The model under review builds one solid part; all positions refer to its coordinate system, in mm. Face numbers are marked on the shaded views. A direction names the side the tool comes from. Coordinates: 2 decimals unless noted, no trailing zeros. Order: outer loops, then holes, each group sorted by start corner. A loop starts at its lowest first (then second) coordinate and runs counter-clockwise, first axis right, second up. Notation, with made-up numbers: M 27.25,4.25 L 38.25,4.25 A33 cw 38.25,43.25 Z; hole C -37.75,70 d1. An arc over 180 degrees is marked long. Answer in a Markdown table with one row per item.
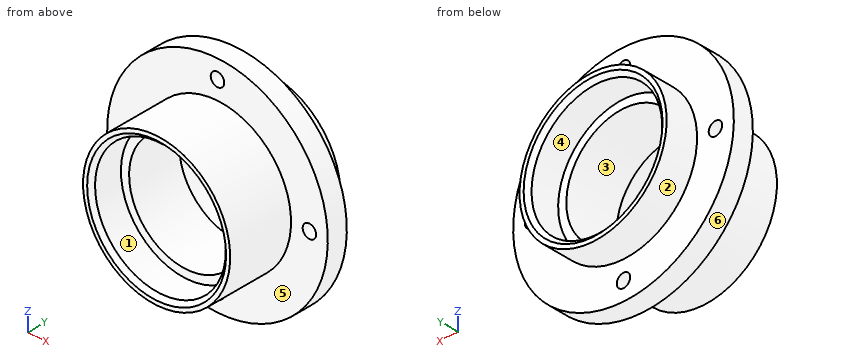
from build123d import *

# Parameters (mm, degrees)
SKETCH1_R             = 18
BOSS_EXTRUDE1_DEPTH   = 8
CUT_EXTRUDE1_REACH    = 28.683
SKETCH2_R             = 16
SKETCH3_R             = 27
BOSS_EXTRUDE2_DEPTH   = 5
BOSS_EXTRUDE3_START   = 16
SKETCH4_R             = 18
BOSS_EXTRUDE3_DEPTH   = 16
SKETCH5_R             = 16
CUT_EXTRUDE2_DEPTH    = 7.8
SKETCH6_R             = 14
CUT_EXTRUDE3_DEPTH    = 44.577517139
M4_TAPPED_HOLE1_D     = 3.3
M4_TAPPED_HOLE1_DEPTH = 11.5
M4_TAPPED_HOLE1_TIP   = 0.991420021
CHAMFER1_SIZE         = 1


with BuildPart() as part:
    # Sketch1 → Boss-Extrude1 (new body)
    with BuildSketch(Plane(origin=(0, 0, 0), x_dir=(1, 0, 0), z_dir=(0, 1, 0))):
        with Locations(Location((0, 0, 0), (0, 0, 270))):
            Circle(SKETCH1_R)
    extrude(amount=BOSS_EXTRUDE1_DEPTH)

    # Sketch2 → Cut-Extrude1 (cut, up to next)
    with BuildSketch(Plane.XZ, mode=Mode.PRIVATE) as cut_extrude1_sk1:
        with Locations(Location((0, 0, 0), (0, 0, 270))):
            Circle(SKETCH2_R)
    cut_extrude1_tool1 = extrude(cut_extrude1_sk1.sketch, amount=-CUT_EXTRUDE1_REACH, mode=Mode.PRIVATE) & part.part
    add(cut_extrude1_tool1.solids().sort_by_distance((0, 0, 0))[0], mode=Mode.SUBTRACT)

    # Sketch3 → Boss-Extrude2 (add)
    with BuildSketch(Plane.XZ):
        with Locations(Location((0, 0, 0), (0, 0, 270))):
            Circle(SKETCH3_R)
    extrude(amount=BOSS_EXTRUDE2_DEPTH)

    # Sketch4 → Boss-Extrude3 (add)
    with BuildSketch(Plane.XZ.offset(5).offset(BOSS_EXTRUDE3_START)):
        with Locations(Location((0, 0, 0), (0, 0, 270))):
            Circle(SKETCH4_R)
    extrude(amount=-BOSS_EXTRUDE3_DEPTH)

    # Sketch5 → Cut-Extrude2 (cut)
    with BuildSketch(Plane.XZ.offset(21)):
        with Locations(Location((0, 0, 0), (0, 0, 270))):
            Circle(SKETCH5_R)
    extrude(amount=-CUT_EXTRUDE2_DEPTH, mode=Mode.SUBTRACT)

    # Sketch6 → Cut-Extrude3 (cut, through all)
    with BuildSketch(Plane(origin=(0, 0, 0), x_dir=(1, 0, 0), z_dir=(0, 1, 0))):
        with Locations(Location((0, 0, 0), (0, 0, 270))):
            Circle(SKETCH6_R)
    extrude(amount=-CUT_EXTRUDE3_DEPTH, mode=Mode.SUBTRACT)

    # M4 Tapped Hole1
    with Locations(Plane(origin=(0, 0, 0), x_dir=(1, 0, 0), z_dir=(0, 1, 0))):
        with Locations((-22.5, 0), (0, 0), (0, 22.5), (22.5, 0), (0, -22.5)):
            Hole(M4_TAPPED_HOLE1_D / 2, depth=M4_TAPPED_HOLE1_DEPTH)
            with Locations((0, 0, -(M4_TAPPED_HOLE1_DEPTH + M4_TAPPED_HOLE1_TIP / 2))):  # 118° drill point
                Cone(0, M4_TAPPED_HOLE1_D / 2, M4_TAPPED_HOLE1_TIP, mode=Mode.SUBTRACT)

    # Chamfer1
    chamfer1_edges = [part.edges().sort_by_distance(p)[0] for p in [
        (0, -21, 16),
        (0, 8, 16),
    ]]
    chamfer(chamfer1_edges, length=CHAMFER1_SIZE)


solid = part.part
(1) To check wall thickness, follow line 1 (Y direction, x = 18, z = 2.5); line 2 (X direction, y = 2.5, z = 10); line 3 (X direction, y = -14.5, z = 0). State the ranges of each line that lie inside material, in increasing order. Write a range as [from, to].
Report:
| item | result |
|---|---|
| line 1 | [-5, 0] |
| line 2 | [-14.97, -12.49], [12.49, 14.97] |
| line 3 | [-18, -16], [16, 18] |
(2) The part is to be moulded in two halves that separate along X. For the marked faces 4, 5 and 6, say which applies: +X half, -X half, draft (parallel to the pull), parting line (faces both ways), or undercut.
Report:
| item | result |
|---|---|
| face 4 | undercut |
| face 5 | draft |
| face 6 | parting line |
(3) Take a section at C-C (z = -22.5). Write out the cut boundary in (x, y), then the cut area to 3 significant figures.
Report:
| item | result |
|---|---|
| outline | M -14.92,-5 L -1.65,-5 L -1.65,0 L -14.92,0 Z; M 1.65,-5 L 14.92,-5 L 14.92,0 L 1.65,0 Z |
| area | 133 mm^2 |
(4) Machinability: for the marked faces 1, 2 and 3, which of the approach directions +Z, -Z, +X, -X, +Y, -Y give a long, thin tool a straight path to every point of the face, cutting with its end or side? Answer none if there is none.
Report:
| item | result |
|---|---|
| face 1 | -Y |
| face 2 | +Y |
| face 3 | +Y, -Y |
(5) Take a section at D-D (y = -10.5). Write out the cut boundary in (x, z), then the cut area to 3 significant figures.
Report:
| item | result |
|---|---|
| outline | C 0,0 d36; hole C 0,0 d28 |
| area | 402 mm^2 |
(6) Take a section at B-B (x = -23). Write out the cut boundary in (y, z), then the cut area to 3 significant figures.
Report:
| item | result |
|---|---|
| outline | M -5,-14.14 L 0,-14.14 L 0,-1.57 L -5,-1.57 Z; M -5,1.57 L 0,1.57 L 0,14.14 L -5,14.14 Z |
| area | 126 mm^2 |
(7) Take a section at A-A (y = -2). Write out the cut boundary in (x, z).
Report:
| item | result |
|---|---|
| outline | C 0,0 d54; hole C -22.5,0 d3.3; hole C 0,0 d28; hole C 0,-22.5 d3.3; hole C 0,22.5 d3.3; hole C 22.5,0 d3.3 |
(8) Insertion check: P1, Ø1, axis at x = 6.5, y = -12.5, coming from the -Z side; P2, Ø8, axis at x = -2.5, y = -10.5, coming from the +Z side; P3, Ø4, axis at x = 0, z = 22.5, coming from the -Y side. Each pin has a flat end and moves straight along its axis. Give the tip position at first contact, or say it passes through.
Report:
| item | result |
|---|---|
| P1 | z = -16.97 |
| P2 | z = 18 |
| P3 | y = -5 |
